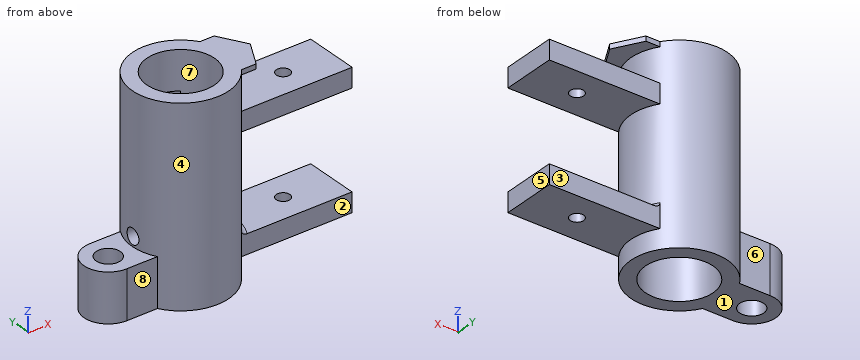
from build123d import *

# Parameters (mm, degrees)
BODY_PROFILE_100_R         = 50
HOUSING_BODY_100X200_DEPTH = 200
FRONT_BORE_PROFILE_70_R    = 35
FRONT_BORE_70X40_DEPTH     = 40
INNER_RECESS_PROFILE_75_R  = 37.5
INNER_RECESS_75X80_DEPTH   = 80
THROUGH_BORE_PROFILE_70_R  = 35
THROUGH_BORE_70_DEPTH      = 213.132034356
REAR_START                 = -5
REAR_TAB_5MM_DEPTH         = 5
LUG_PLATES_DEPTH           = 20
LUG_WEB_PROFILE_W          = 114.575369646
LUG_WEB_PROFILE_H          = 56
LUG_WEB_DEPTH              = 20
LUG_PIN_HOLES_PROFILE_14_R = 7
LUG_PIN_HOLES_14_DEPTH     = 229.989082709
LUG_WEB_FILLET_R5_R        = 5
TOP_BOSS_PROFILE_R         = 12.5
TOP_BOSS_DEPTH             = 50
TOP_BOSS_HOLE_PROFILE_16_R = 8
TOP_BOSS_HOLE_16_DEPTH     = 50


with BuildPart() as part:
    # Body Profile Ø100 → Housing Body Ø100x200 (new body)
    with BuildSketch(Plane.XY):
        Circle(BODY_PROFILE_100_R)
    extrude(amount=HOUSING_BODY_100X200_DEPTH)

    # Front Bore Profile Ø70 → Front Bore Ø70x40 (cut)
    with BuildSketch(Plane.XY.offset(200)):
        Circle(FRONT_BORE_PROFILE_70_R)
    extrude(amount=-FRONT_BORE_70X40_DEPTH, mode=Mode.SUBTRACT)

    # Inner Recess Profile Ø75 → Inner Recess Ø75x80 (cut)
    with BuildSketch(Plane.XY.offset(160)):
        Circle(INNER_RECESS_PROFILE_75_R)
    extrude(amount=-INNER_RECESS_75X80_DEPTH, mode=Mode.SUBTRACT)

    # Through Bore Profile Ø70 → Through Bore Ø70 (cut, through all)
    with BuildSketch(Plane(origin=(0, 0, 0), x_dir=(-1, 0, 0), z_dir=(0, 0, -1))):
        with Locations(Location((0, 0, 0), (0, 0, 180))):
            Circle(THROUGH_BORE_PROFILE_70_R)
    extrude(amount=-THROUGH_BORE_70_DEPTH, mode=Mode.SUBTRACT)

    # Rear Tab Profile → Rear Tab 5mm (add)
    with BuildSketch(Plane.XY.offset(200).offset(REAR_START)):
        with BuildLine():
            Line((72, 0), (56, 28))
            Line((56, 28), (41.424630354, 28))
            ThreePointArc((41.424630354, 28), (50, 0), (41.424630354, -28))
            Line((41.424630354, -28), (56.712315177, -28))
            Line((56.712315177, -28), (72, 0))
        make_face()
    extrude(amount=REAR_TAB_5MM_DEPTH)

    # Lug Plates Profile → Lug Plates (add)
    with BuildSketch(Plane.XY.offset(140)):
        with BuildLine():
            Line((21, -28), (156, -28))
            Line((156, -28), (156, 28))
            Line((156, 28), (21, 28))
            ThreePointArc((21, 28), (35, 0), (21, -28))
        make_face()
    extrude(amount=LUG_PLATES_DEPTH)

    # Lug Web Profile → Lug Web (add)
    with BuildSketch(Plane.XY.offset(20)):
        with Locations((98.712315177, 0)):
            Rectangle(LUG_WEB_PROFILE_W, LUG_WEB_PROFILE_H)
    extrude(amount=LUG_WEB_DEPTH)

    # Lug Pin Holes Profile Ø14 → Lug Pin Holes Ø14 (cut, through all)
    with BuildSketch(Plane.XY.offset(160)):
        with Locations(Location((106, 0, 0), (0, 0, 180))):
            Circle(LUG_PIN_HOLES_PROFILE_14_R)
    extrude(amount=-LUG_PIN_HOLES_14_DEPTH, mode=Mode.SUBTRACT)

    # Lug Web Fillet R5
    lug_web_fillet_r5_edges = [part.edges().sort_by_distance(p)[0] for p in [
        (47.808113944, -14.64186604, 40),
    ]]
    fillet(lug_web_fillet_r5_edges, radius=LUG_WEB_FILLET_R5_R)

    # Top Boss Profile → Top Boss (add)
    with BuildSketch(Plane.XY):
        with BuildLine():
            Line((-75, 25), (-43.301270189, 25))
            ThreePointArc((-43.301270189, 25), (-50, 0), (-43.301270189, -25))
            Line((-43.301270189, -25), (-75, -25))
            ThreePointArc((-75, -25), (-100, 0), (-75, 25))
        make_face()
        with Locations((-75, 0)):
            Circle(TOP_BOSS_PROFILE_R, mode=Mode.SUBTRACT)
    extrude(amount=TOP_BOSS_DEPTH)

    # Top Boss Hole Profile Ø16 → Top Boss Hole Ø16 (cut)
    with BuildSketch(Plane(origin=(-50, 0, 0), x_dir=(0, 0, -1), z_dir=(1, 0, 0))):
        with Locations(Location((-60, 0, 0), (0, 0, 180))):
            Circle(TOP_BOSS_HOLE_PROFILE_16_R)
    extrude(amount=TOP_BOSS_HOLE_16_DEPTH, mode=Mode.SUBTRACT)


solid = part.part
Build history of the part. All positions in model axes, mm. Face numbers are marked on the shaded views. A direction names the side the tool comes from. Round coordinates to 2 decimals unless told otherwise and drop trailing zeros. Loops run counter-clockwise (first coordinate to the right, second up) from the corner with the lowest first, then second, coordinate; pieces in that order, holes last. Notation, with made-up numbers: (1, 12.25) -> (26, 12.25) arc R37 cw to (26, 49.25) -> close; hole circle Ø4 at (19.5, 85). An arc over 180 degrees is marked (long way). Answer in a Markdown table with one row per item.
Item 1: Pin check, flat tips, straight feed: pin 1 (5 mm diameter, centred on x = 70, z = 155, fed in from +Y); pin 2 (4 mm diameter, centred on y = 27.5, z = 54, fed in from +X); pin 3 (1.5 mm diameter, centred on x = 52, z = 145, fed in from -Y); pin 4 (11 mm diameter, centred on x = 106, y = 0, fed in from +Z). Stop position of each tip, or through.
Answers below:
| item | result |
|---|---|
| pin 1 | stops at y = 28 |
| pin 2 | stops at x = 43.01 |
| pin 3 | stops at y = -28 |
| pin 4 | passes through |
Item 2: Drill centre lines: L1, parallel to Z at x = 65.5, y = 3; L2, parallel to Y at x = 0, z = 55.5; L3, parallel to Z at x = 132.5, y = -21.5. Where is each one in solid material? Low to high. Write a range as [from, to].
Answers below:
| item | result |
|---|---|
| L1 | z = [20, 40], [140, 160], [195, 200] |
| L2 | y = [-50, -35], [35, 50] |
| L3 | z = [20, 40], [140, 160] |
Item 3: Saw through at B-B (x = 106). Write the cut outline in (y, z), and give its area (3 significant figures).
Answers below:
| item | result |
|---|---|
| outline | (-28, 20) -> (-7, 20) -> (-7, 40) -> (-28, 40) -> close; (-28, 140) -> (-7, 140) -> (-7, 160) -> (-28, 160) -> close; (7, 20) -> (28, 20) -> (28, 40) -> (7, 40) -> close; (7, 140) -> (28, 140) -> (28, 160) -> (7, 160) -> close |
| area | 1,680 mm² |
Item 4: Which spindle directions (+Z, -Z, +X, -X, +Y, -Y) get a long thin tool onto all of the face, cutting with end or side? Do the marked faces 1, 2, 3 and 4. Say none if no direction does.
Answers below:
| item | result |
|---|---|
| face 1 | -Z, +X, -X, +Y, -Y |
| face 2 | +Z, -Z, +X, -Y |
| face 3 | +Z, -Z, +X, +Y |
| face 4 | none |
Item 5: Saw through at D-D (z = 188). Write the cut outline in (x, y).
Answers below:
| item | result |
|---|---|
| outline | circle Ø100 at (0, 0); hole circle Ø70 at (0, 0) |
Item 6: Saw through at A-A (x = 0). Write the cut outline in (y, z).
Answers below:
| item | result |
|---|---|
| outline | (-50, 0) -> (-35, 0) -> (-35, 80) -> (-37.5, 80) -> (-37.5, 160) -> (-35, 160) -> (-35, 200) -> (-50, 200) -> close; (35, 0) -> (50, 0) -> (50, 200) -> (35, 200) -> (35, 160) -> (37.5, 160) -> (37.5, 80) -> (35, 80) -> close |
Item 7: Mould opens along Y. For the marked faces 5, 6, 7 and 8 say: +Y half, -Y half, draft (parallel to the pull), parting line (faces both ways), or undercut.
Answers below:
| item | result |
|---|---|
| face 5 | draft |
| face 6 | +Y half |
| face 7 | undercut |
| face 8 | -Y half |
Item 8: Saw through at C-C (z = 104). Write the cut outline in (x, y), and give its area (3 significant figures).
Answers below:
| item | result |
|---|---|
| outline | circle Ø100 at (0, 0); hole circle Ø75 at (0, 0) |
| area | 3,440 mm² |
